Geometry check sheet. Reference: the model listing, model coordinates, mm. Face numbers are marked on the shaded views. A direction names the side the tool comes from. Give positions to 0.01 mm unless a question says otherwise; leave off trailing zeros. Loops run counter-clockwise (first coordinate to the right, second up) from the corner with the lowest first, then second, coordinate; pieces in that order, holes last. Notation, with made-up numbers: (88, 36) -> (136, 36) arc R29 cw to (136, 75) -> close; hole circle Ø1 at (-36, -9). An arc over 180 degrees is marked (long way). Answer in a Markdown table with one row per item. Add a question column.
```python
from build123d import *

# Parameters (mm, degrees)
BOSS_EXTRUDE2_DEPTH = 6
SKETCH3_R           = 4.5
BOSS_EXTRUDE3_DEPTH = 15


with BuildPart() as part:
    # Sketch2 → Boss-Extrude2 (new body)
    with BuildSketch(Plane.XY):
        Polygon((0, 9.237604307), (-8, 4.618802154), (-8, -4.618802154), (0, -9.237604307), (8, -4.618802154), (8, 4.618802154), align=None)
    extrude(amount=BOSS_EXTRUDE2_DEPTH)

    # Sketch3 → Boss-Extrude3 (add)
    with BuildSketch(Plane.XY.offset(6)):
        Circle(SKETCH3_R)
    extrude(amount=BOSS_EXTRUDE3_DEPTH)


solid = part.part
```
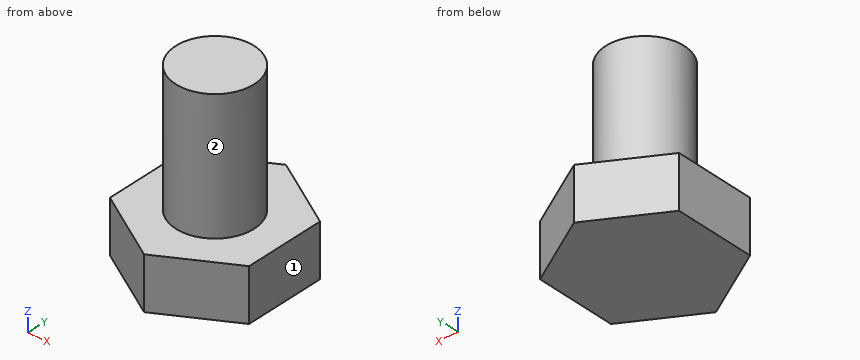
1. Sectioned sample at D-D (z = 19.5). Enter the section's corners in (x, y).
2. Sectioned sample at A-A (y = 0). Enter the section's corners in (x, z).
3. Gauge pin test, flat ends, axial feed: pin 1 Ø1.5 at (y, z) = (6.5, 6) entering from +X; pin 2 Ø8 at (x, z) = (3, 7.5) entering from +Y; pin 3 Ø6 at (y, z) = (6, 11.5) entering from -X; pin 4 Ø4 at (y, z) = (-1.5, 12) entering from -X. Record the tip position at first contact, or that the pin passes through.
4. Sectioned sample at B-B (x = -3.25). Enter the section's corners in (y, z).
5. Sectioned sample at C-C (z = 3). Enter the section's corners in (x, y), plus the area to 3 significant figures.
6. Material ranges on L1, parallel to Z at x = 2, y = 5.25; L2, parallel to X at y = 3.25, z = 6.5; L3, parallel to X at y = -1, z = 19.5, recorded low to high. Write a range as from..to.
7. Access from +Z, -Z, +X, -X, +Y, -Y to the whole of each face (thin tool, end or side, straight path). Record for the marked faces 1 and 2.
Response:
| question | item | result |
|---|---|---|
| 1 | outline | circle Ø9 at (0, 0) |
| 2 | outline | (-8, 0) -> (8, 0) -> (8, 6) -> (4.5, 6) -> (4.5, 21) -> (-4.5, 21) -> (-4.5, 6) -> (-8, 6) -> close |
| 3 | pin 1 | stops at x = 6.04 |
| 3 | pin 2 | stops at y = 9.24 |
| 3 | pin 3 | stops at x = -3.35 |
| 3 | pin 4 | stops at x = -4.5 |
| 4 | outline | (-7.36, 0) -> (7.36, 0) -> (7.36, 6) -> (3.11, 6) -> (3.11, 21) -> (-3.11, 21) -> (-3.11, 6) -> (-7.36, 6) -> close |
| 5 | outline | (-8, -4.62) -> (0, -9.24) -> (8, -4.62) -> (8, 4.62) -> (0, 9.24) -> (-8, 4.62) -> close |
| 5 | area | 222 mm2 |
| 6 | L1 | z = 0..6 |
| 6 | L2 | x = -3.11..3.11 |
| 6 | L3 | x = -4.39..4.39 |
| 7 | face 1 | +Z, -Z, +X, +Y, -Y |
| 7 | face 2 | +Z |
